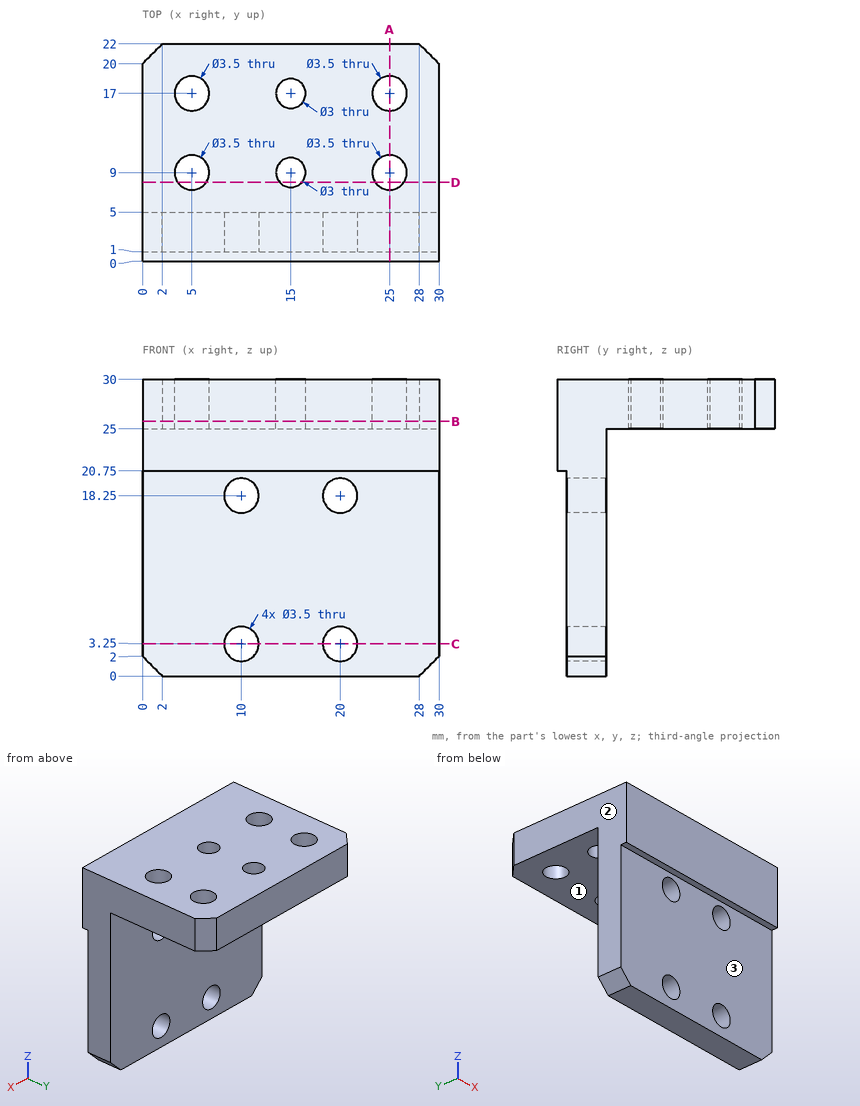
Could you check a few things on this drawing? It's one solid part, dimensions in mm from its lowest x, y, z. A direction names the side the tool comes from. Round coordinates to 2 decimals unless told otherwise and drop trailing zeros. Loops run counter-clockwise (first coordinate to the right, second up) from the corner with the lowest first, then second, coordinate; pieces in that order, holes last. Notation, with made-up numbers: (59, -25) -> (98, -25) arc R30 cw to (98, 13) -> close; hole circle Ø11 at (-20, -29). An arc over 180 degrees is marked (long way). One line per item, written item: value. Start each with the question number.
1. For the marked faces 1, 2 and 3, which set-ups out of +Z, -Z, +X, -X, +Y, -Y let a thin tool reach every point of the face, with its end or its side?
2. If we section it at D-D, the plane y = 8: Write out the boundary of the cut face in (x, z).
3. For pin 1 (5.5 mm diameter, centred on x = 25, y = 9, fed in from +Z); pin 2 (3 mm diameter, centred on x = 12, z = 3, fed in from -Y); pin 3 (4.5 mm diameter, centred on x = 5, y = 17, fed in from -Z); pin 4 (5.5 mm diameter, centred on x = 20, z = 3.25, fed in from +Y), each with a flat end and sliding along its axis, tell me the tip position at first contact or that it passes through.
4. If I drill on probe 1 along Y at (x, z) = (25, 26.8); probe 2 along X at (y, z) = (2.7, 18.25); probe 3 along Z at (x, y) = (13.75, 10), over which ranges is the centre line in solid material (lowest first)?
5. If we section it at C-C, the plane z = 3.25: Write out the boundary of the cut face in (x, y), then the cut area to 3 significant figures.
6. If we section it at B-B, the plane z = 25.75: Write out the boundary of the cut face in (x, y), then the cut area to 3 significant figures.
7. If we section it at A-A, the plane x = 25: Write out the boundary of the cut face in (y, z).
Calculated:
1. face 1: -Z, +X, -X, +Y
1. face 2: +Z, -Z, -X, +Y, -Y
1. face 3: -Z, +X, -X, -Y
2. outline: (0, 25) -> (3.56, 25) -> (3.56, 30) -> (0, 30) -> close; (6.44, 25) -> (13.88, 25) -> (13.88, 30) -> (6.44, 30) -> close; (16.12, 25) -> (23.56, 25) -> (23.56, 30) -> (16.12, 30) -> close; (26.44, 25) -> (30, 25) -> (30, 30) -> (26.44, 30) -> close
3. pin 1: stops at z = 30
3. pin 2: stops at y = 1
3. pin 3: stops at z = 25
3. pin 4: stops at y = 5
4. probe 1: y = 0 to 7.25, 10.75 to 15.25, 18.75 to 22
4. probe 2: x = 0 to 8.25, 11.75 to 18.25, 21.75 to 30
4. probe 3: z = 25 to 30
5. outline: (0, 1) -> (8.25, 1) -> (8.25, 5) -> (0, 5) -> close; (11.75, 1) -> (18.25, 1) -> (18.25, 5) -> (11.75, 5) -> close; (21.75, 1) -> (30, 1) -> (30, 5) -> (21.75, 5) -> close
5. area: 92.0 mm²
6. outline: (0, 0) -> (30, 0) -> (30, 20) -> (28, 22) -> (2, 22) -> (0, 20) -> close; hole circle Ø3.5 at (5, 9); hole circle Ø3.5 at (5, 17); hole circle Ø3 at (15, 9); hole circle Ø3 at (15, 17); hole circle Ø3.5 at (25, 9); hole circle Ø3.5 at (25, 17)
6. area: 603 mm²
7. outline: (0, 20.75) -> (1, 20.75) -> (1, 0) -> (5, 0) -> (5, 25) -> (7.25, 25) -> (7.25, 30) -> (0, 30) -> close; (10.75, 25) -> (15.25, 25) -> (15.25, 30) -> (10.75, 30) -> close; (18.75, 25) -> (22, 25) -> (22, 30) -> (18.75, 30) -> close
